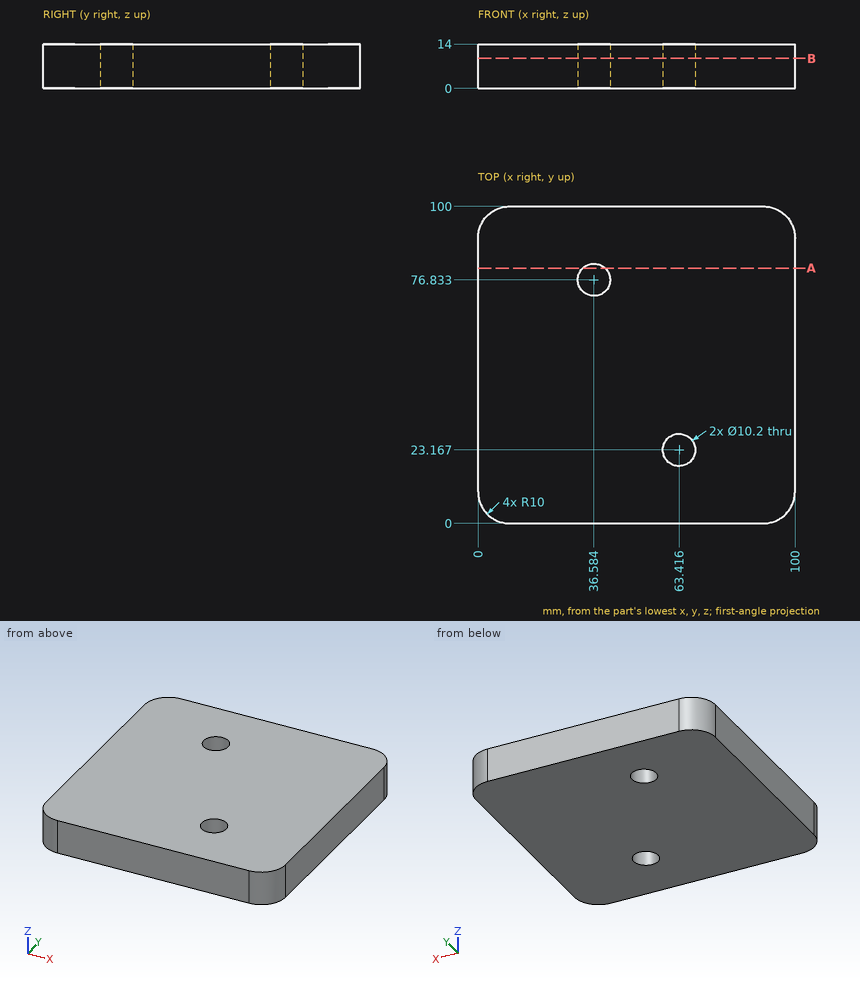
Could you check a few things on this drawing? It's one solid part, dimensions in mm from its lowest x, y, z. Coordinates: 2 decimals unless noted, no trailing zeros. Write each loop counter-clockwise with the first axis right and the second up, starting at its lowest first coordinate (ties: lowest second). Pieces come first, ordered by that corner, then holes. Notation, with made-up numbers: (79, 86.5) - (135, 86.5) arc R16 cw to (135, 104.5) - close; hole circle Ø1 at (-9, 38.5). An arc over 180 degrees is marked (long way). Put each result on its own line as item: value. Start each with the question number.
Q1. I want a section at A-A on y = 80.5. Write out the boundary of the cut face in (x, z), plus the area to 3 significant figures.
Q2. I want a section at B-B on z = 9.5. Write out the boundary of the cut face in (x, y), plus the area to 3 significant figures.
Q3. Please list where these lines run through material, in increasing order: L1, parallel to X at y = 79.5, z = 8.25 (1 decimal); L2, parallel to Y at x = 65, z = 6.25 (1 decimal); L3, parallel to X at y = 76, z = 9 (1 decimal).
Checks:
1. outline: (0, 0) - (33.04, 0) - (33.04, 14) - (0, 14) - close; (40.13, 0) - (100, 0) - (100, 14) - (40.13, 14) - close
1. area: 1,300 mm²
2. outline: (0, 10) arc R10 ccw to (10, 0) - (90, 0) arc R10 ccw to (100, 10) - (100, 90) arc R10 ccw to (90, 100) - (10, 100) arc R10 ccw to (0, 90) - close; hole circle Ø10.2 at (36.58, 76.83); hole circle Ø10.2 at (63.42, 23.17)
2. area: 9,750 mm²
3. L1: 0 to 32.2, 40.9 to 100
3. L2: 0 to 18.3, 28 to 100
3. L3: 0 to 31.6, 41.6 to 100
